Model file for the job. Use its own axes, mm. A direction names the side the tool comes from. Coordinates: 2 decimals unless noted, no trailing zeros. Order: outer loops, then holes, each group sorted by start corner. A loop starts at its lowest first (then second) coordinate and runs counter-clockwise, first axis right, second up. Notation, with made-up numbers: (78.25, 78.25) - (113.25, 78.25) arc R16 cw to (113.25, 92.25) - close; hole circle Ø3 at (-31, 74.5). An arc over 180 degrees is marked (long way). Put each result on its own line as item: value. Start each with the question number.
```python
from build123d import *

# Parameters (mm, degrees)
SKETCH_1_R      = 6
EXTRUDE_1_DEPTH = 10


with BuildPart() as part:
    # 草图1 → 凸台-拉伸1 (new body)
    with BuildSketch(Plane.XY):
        with BuildLine():
            Line((130, 208), (130, 58))
            Line((130, 58), (0, 0))
            Line((0, 0), (0, 208))
            Line((0, 208), (25, 208))
            Line((25, 208), (25, 168))
            ThreePointArc((25, 168), (65, 128), (105, 168))
            Line((105, 168), (105, 208))
            Line((105, 208), (130, 208))
        make_face()
        with Locations((117.5, 168)):
            Circle(SKETCH_1_R, mode=Mode.SUBTRACT)
        with Locations((12.5, 168)):
            Circle(SKETCH_1_R, mode=Mode.SUBTRACT)
        with Locations((40, 43.72)):
            Circle(SKETCH_1_R, mode=Mode.SUBTRACT)
        with Locations((90, 65.43)):
            Circle(SKETCH_1_R, mode=Mode.SUBTRACT)
    extrude(amount=EXTRUDE_1_DEPTH)


solid = part.part
```
Item 1: Slice it at C-C, the plane x = 40. Give the cut face in (y, z), plus the area to 3 significant figures.
Item 2: Wall check: line 1 along X through (y, z) = (66, 8); line 2 along Y through (x, z) = (89, 7.5); line 3 along X through (y, z) = (148, 0.5). Give the ranges that are in metal, low to high.
Item 3: Pull direction X, two halves, no side cores. Call faces 3 (the face through (64.12, 128.01, 4.93)), 4 (the face through (65.9, 29.4, 4.9)), 5 (the face through (12, 208, 5)): pulls with the +X half, pulls with the -X half, needs draft (parallel to the pull), parting line crosses it, or undercut.
Item 4: Slice it at A-A, the plane y = 65.43. Give the cut face in (x, z).
Item 5: Slice it at B-B, the plane z = 7.5. Give the cut face in (x, y).
Item 6: Slice it at D-D, the plane x = 65. Give the cut face in (y, z).
Item 7: 3-axis set-ups, long thin cutter, end or side, ignore diameter. For faces 1 (the face through (0, 103, 5)), 2 (the face through (105, 188, 5)): which of +Z, -Z, +X, -X, +Y, -Y reach the whole face in a straight line?
Item 8: Flat gauge pins, fed straight in: pin 1 Ø7 at (x, y) = (117.5, 168) entering from -Z; pin 2 Ø12 at (x, y) = (100, 61.5) entering from -Z; pin 3 Ø3 at (x, z) = (36.5, 7.5) entering from +Y; pin 4 Ø2 at (x, z) = (28, 2) entering from -Y. Where does each tip first touch, or does it go through?
Here are the results:
1. outline: (17.85, 0) - (37.72, 0) - (37.72, 10) - (17.85, 10) - close; (49.72, 0) - (136.78, 0) - (136.78, 10) - (49.72, 10) - close
1. area: 1,070 mm^2
2. line 1: x = 0 to 84.03, 95.97 to 130
2. line 2: y = 39.71 to 59.51, 71.35 to 136
2. line 3: x = 0 to 30.36, 99.64 to 130
3. face 3: undercut
3. face 4: pulls with the +X half
3. face 5: needs draft
4. outline: (0, 0) - (84, 0) - (84, 10) - (0, 10) - close; (96, 0) - (130, 0) - (130, 10) - (96, 10) - close
5. outline: (0, 0) - (130, 58) - (130, 208) - (105, 208) - (105, 168) arc R40 cw to (25, 168) - (25, 208) - (0, 208) - close; hole circle Ø12 at (12.5, 168); hole circle Ø12 at (40, 43.72); hole circle Ø12 at (90, 65.43); hole circle Ø12 at (117.5, 168)
6. outline: (29, 0) - (128, 0) - (128, 10) - (29, 10) - close
7. face 1: +Z, -Z, -X, +Y, -Y
7. face 2: +Z, -Z, +Y
8. pin 1: passes through
8. pin 2: stops at z = 0
8. pin 3: stops at y = 141.54
8. pin 4: stops at y = 12.05
